```python
from build123d import *

# Parameters (mm, degrees)
SKETCH_1_W          = 500
SKETCH_1_H          = 300
EXTRUDE_1_DEPTH     = 45
CHAMFER_1_SIZE      = 5
SKETCH_6_R          = 40
CUT_EXTRUDE_1_DEPTH = 296
HOLE_WIZARD_M10_3_D = 8.5
HOLE_WIZARD_M8_1_D  = 6.8


with BuildPart() as part:
    # 草图1 → 凸台-拉伸1 (new body)
    with BuildSketch(Plane(origin=(0, 0, 0), x_dir=(1, 0, 0), z_dir=(0, 1, 0))):
        Rectangle(SKETCH_1_W, SKETCH_1_H)
    extrude(amount=EXTRUDE_1_DEPTH)

    # 倒角1
    chamfer_1_edges = [part.edges().sort_by_distance(p)[0] for p in [
        (250, 22.5, 150),
        (-250, 22.5, 150),
        (-250, 22.5, -150),
        (250, 22.5, -150),
    ]]
    chamfer(chamfer_1_edges, length=CHAMFER_1_SIZE)

    # 草图6 → 切除-拉伸1 (cut, through all)
    with BuildSketch(Plane(origin=(0, 45, 0), x_dir=(1, 0, 0), z_dir=(0, 1, 0))):
        with Locations(Location((190, -90, 0), (0, 0, 270))):
            Circle(SKETCH_6_R)
        with Locations(Location((190, 90, 0), (0, 0, 270))):
            Circle(SKETCH_6_R)
        with Locations(Location((-190, 90, 0), (0, 0, 270))):
            Circle(SKETCH_6_R)
        with Locations(Location((-190, -90, 0), (0, 0, 270))):
            Circle(SKETCH_6_R)
    extrude(amount=-CUT_EXTRUDE_1_DEPTH, mode=Mode.SUBTRACT)

    # M10 螺纹孔3 (through all)
    with Locations(Plane(origin=(0, 45, 0), x_dir=(1, 0, 0), z_dir=(0, 1, 0))):
        with Locations((-12.293904642, 45.881476749), (-45.881476749, 12.293904642), (-33.587572106, -33.587572106), (12.293904642, -45.881476749), (45.881476749, -12.293904642), (33.587572106, 33.587572106)):
            Hole(HOLE_WIZARD_M10_3_D / 2)

    # M8 螺纹孔1 (through all)
    with Locations(Plane(origin=(0, 45, 0), x_dir=(1, 0, 0), z_dir=(0, 1, 0))):
        with Locations((239, -90), (190, -139), (141, -90), (190, -41), (239, 90), (190, 41), (141, 90), (190, 139), (-141, -90), (-190, -139), (-239, -90), (-190, -41), (-141, 90), (-190, 41), (-239, 90), (-190, 139)):
            Hole(HOLE_WIZARD_M8_1_D / 2)


solid = part.part
```
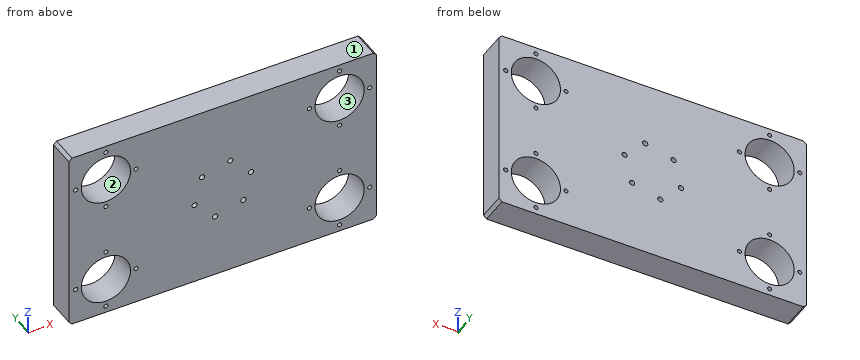
Geometry check sheet. Reference: the model listing, model coordinates, mm. Face numbers are marked on the shaded views. Round coordinates to 2 decimals unless told otherwise and drop trailing zeros. Write each loop counter-clockwise with the first axis right and the second up, starting at its lowest first coordinate (ties: lowest second). Pieces come first, ordered by that corner, then holes. Notation, with made-up numbers: (53, -2.75) -> (105, -2.75) arc R19 cw to (105, 13.25) -> close; hole circle Ø8 at (86.25, 39). An arc over 180 degrees is marked (long way). Put each result on its own line as item: value.
1) Release check for a two-part mould opening along X. For the marked faces 1, 2 and 3 record: pulls with the +X half, pulls with the -X half, needs draft (parallel to the pull), parting line crosses it, or undercut.
Recorded:
face 1: needs draft
face 2: undercut
face 3: undercut
2) Thickness scan on probe 1 along Z at (x, y) = (239, 25); probe 2 along X at (y, z) = (27, 139); probe 3 along Z at (x, y) = (-222.5, 36). Record the ranges inside material, lowest first. Write a range as from..to.
Recorded:
probe 1: z = -150..-93.4, -86.6..86.6, 93.4..150
probe 2: x = -250..-193.4, -186.6..186.6, 193.4..250
probe 3: z = -150..-113.32, -66.68..66.68, 113.32..150
3) Cross-section at C-C, the plane y = 11. Give the number of separate pieces and of enclosed holes in the cut face, plus the area to 3 significant figures.
Recorded:
separate pieces: 1
enclosed holes: 26
area: 129,000 mm2
4) Cross-section at A-A, the plane z = 119. Enter the section's corners in (x, y), plus the area to 3 significant figures.
Recorded:
outline: (-250, 0) -> (-217.55, 0) -> (-217.55, 45) -> (-250, 45) -> close; (-162.45, 0) -> (162.45, 0) -> (162.45, 45) -> (-162.45, 45) -> close; (217.55, 0) -> (250, 0) -> (250, 45) -> (217.55, 45) -> close
area: 17,500 mm2
5) Cross-section at B-B, the plane x = -159. Enter the section's corners in (y, z), plus the area to 3 significant figures.
Recorded:
outline: (0, -150) -> (45, -150) -> (45, -115.28) -> (0, -115.28) -> close; (0, -64.72) -> (45, -64.72) -> (45, 64.72) -> (0, 64.72) -> close; (0, 115.28) -> (45, 115.28) -> (45, 150) -> (0, 150) -> close
area: 8,950 mm2
